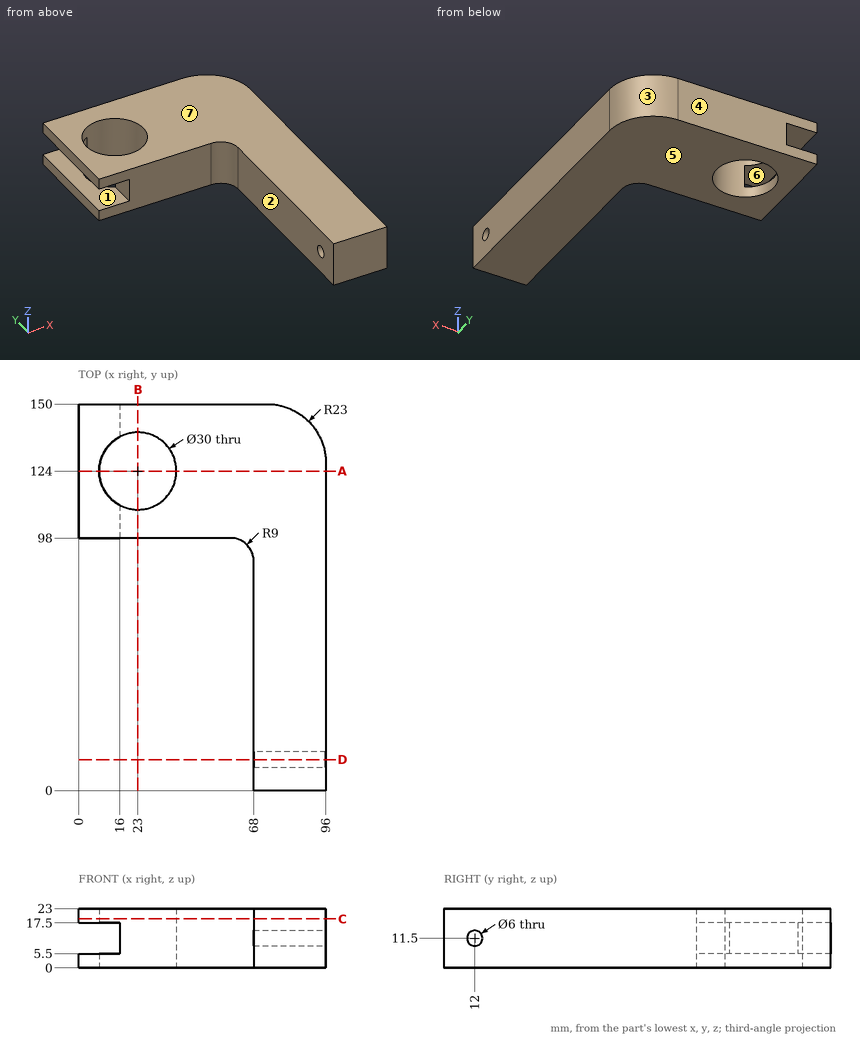
Can you work these out from the drawing? Everything is in mm from the part's minimum corner. A direction names the side the tool comes from. Round coordinates to 2 decimals unless told otherwise and drop trailing zeros. Loops run counter-clockwise (first coordinate to the right, second up) from the corner with the lowest first, then second, coordinate; pieces in that order, holes last. Notation, with made-up numbers: (69.25, -14.5) - (122.25, -14.5) arc R31 cw to (122.25, 13.5) - close; hole circle Ø10 at (19.25, 61.25). An arc over 180 degrees is marked (long way). Answer in a Markdown table with one row per item. Add a question column.
Q1. I want a section at A-A on y = 124. List the corners of the cut face in (x, z) for me.
Q2. For pin 1 Ø7 at (y, z) = (55, 7.5) entering from -X; pin 2 Ø2 at (x, z) = (11, 18.5) entering from -Y; pin 3 Ø6 at (y, z) = (141, 9) entering from -X, each with a flat end and sliding along its axis, tell me the tip position at first contact or that it passes through.
Q3. Which directions (+Z, -Z, +X, -X, +Y, -Y) give clear straight access to the entire face, cutting with the end or side of a thin tool? Please do the marked faces 1, 2 and 3.
Q4. I want a section at C-C on z = 19. List the corners of the cut face in (x, y) for me, and give its area (3 significant figures).
Q5. I want a section at D-D on y = 12. List the corners of the cut face in (x, z) for me.
Q6. I need wall thicknesses on L1, parallel to X at y = 125, z = 1; L2, parallel to Y at x = 23, z = 11; L3, parallel to Z at x = 74.25, y = 12. Which ranges of each line are inside material? Lowest first, please.
Q7. I want a section at B-B on x = 23. List the corners of the cut face in (y, z) for me.
Q8. We'd pull the mould along Z, two halves only. Please class the marked faces 4, 5, 6 and 7: pulls with the +Z half, pulls with the -Z half, needs draft (parallel to the pull), parting line crosses it, or undercut.
A:
| question | item | result |
|---|---|---|
| 1 | outline | (0, 0) - (8, 0) - (8, 5.5) - (0, 5.5) - close; (0, 17.5) - (8, 17.5) - (8, 23) - (0, 23) - close; (38, 0) - (96, 0) - (96, 23) - (38, 23) - close |
| 2 | pin 1 | x = 68 |
| 2 | pin 2 | y = 98 |
| 2 | pin 3 | x = 16 |
| 3 | face 1 | -X, +Y, -Y |
| 3 | face 2 | +Z, -Z, -X, -Y |
| 3 | face 3 | +Z, -Z, +X, +Y |
| 4 | outline | (0, 98) - (59, 98) arc R9 cw to (68, 89) - (68, 0) - (96, 0) - (96, 127) arc R23 ccw to (73, 150) - (0, 150) - close; hole circle Ø30 at (23, 124) |
| 4 | area | 6,930 mm^2 |
| 5 | outline | (68, 0) - (96, 0) - (96, 8.5) - (68, 8.5) - close; (68, 14.5) - (96, 14.5) - (96, 23) - (68, 23) - close |
| 6 | L1 | 0 to 8.03, 37.97 to 96 |
| 6 | L2 | 98 to 109, 139 to 150 |
| 6 | L3 | 0 to 8.5, 14.5 to 23 |
| 7 | outline | (98, 0) - (109, 0) - (109, 23) - (98, 23) - close; (139, 0) - (150, 0) - (150, 23) - (139, 23) - close |
| 8 | face 4 | needs draft |
| 8 | face 5 | pulls with the -Z half |
| 8 | face 6 | undercut |
| 8 | face 7 | pulls with the +Z half |
